```python
from build123d import *

# Parameters (mm, degrees)
SKETCH1_W           = 60
SKETCH1_H           = 30
BOSS_EXTRUDE1_DEPTH = 20
SKETCH2_W           = 37.506064646
SKETCH2_H           = 6.251724505
BOSS_EXTRUDE2_DEPTH = 5
BOSS_EXTRUDE3_DEPTH = 1


with BuildPart() as part:
    # Sketch1 → Boss-Extrude1 (new body)
    with BuildSketch(Plane(origin=(0, 0, 0), x_dir=(1, 0, 0), z_dir=(0, 1, 0))):
        Rectangle(SKETCH1_W, SKETCH1_H)
    extrude(amount=BOSS_EXTRUDE1_DEPTH)

    # Sketch2 → Boss-Extrude2 (add)
    with BuildSketch(Plane(origin=(0, 0, -15), x_dir=(-1, 0, 0), z_dir=(0, 0, -1))):
        with Locations((0, 9.939278845)):
            Rectangle(SKETCH2_W, SKETCH2_H)
    extrude(amount=BOSS_EXTRUDE2_DEPTH)

    # Sketch3 → Boss-Extrude3 (add)
    with BuildSketch(Plane.XZ):
        with BuildLine():
            Line((-30, 7.472956379), (-30, -8.939791774))
            ThreePointArc((-30, -8.939791774), (-38.206374076, -0.733417697), (-30, 7.472956379))
        make_face()
        with BuildLine():
            Line((30, 7.472956379), (30, -8.939791774))
            ThreePointArc((30, -8.939791774), (38.206374076, -0.733417697), (30, 7.472956379))
        make_face()
        with BuildLine():
            Line((-19.626363832, 15), (21.109917151, 15))
            Line((21.109917151, 15), (21.109917151, 16.556070662))
            ThreePointArc((21.109917151, 16.556070662), (19.645451057, 20.091604568), (16.109917151, 21.556070662))
            Line((16.109917151, 21.556070662), (-14.626363832, 21.556070662))
            ThreePointArc((-14.626363832, 21.556070662), (-18.161897738, 20.091604568), (-19.626363832, 16.556070662))
            Line((-19.626363832, 16.556070662), (-19.626363832, 15))
        make_face()
    extrude(amount=-BOSS_EXTRUDE3_DEPTH)


solid = part.part
```
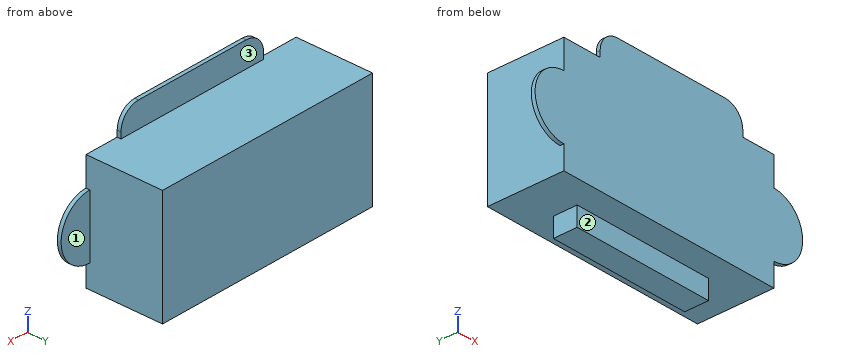
Design review of the part built by this model. Coordinates are the model's own, in mm. Face numbers are marked on the shaded views. A direction names the side the tool comes from. Give positions to 0.01 mm unless a question says otherwise; leave off trailing zeros. Write each loop counter-clockwise with the first axis right and the second up, starting at its lowest first coordinate (ties: lowest second). Pieces come first, ordered by that corner, then holes. Notation, with made-up numbers: (-6, 79) - (24, 79) arc R36 cw to (24, 114) - close; hole circle Ø2 at (-12.5, 75). An arc over 180 degrees is marked (long way). Return JSON: item names as keys, results as strings. Group by question number.
(1) Insertion check: pin 1 (2.5 mm diameter, centred on x = -3.5, z = -17.5, fed in from +Y); pin 2 (6 mm diameter, centred on y = 12.5, z = -4.5, fed in from +X); pin 3 (10 mm diameter, centred on y = 8.5, z = -4.5, fed in from -X). Each pin has a flat end and moves straight along its axis. Give the tip position at first contact, or say it passes through.
(2) We need section A-A, the plane y = 11. Give the boundary of the cut face in (x, z), then the cut area to 3 significant figures.
(3) Machinability: for the marked faces 1, 2 and 3, which of the approach directions +Z, -Z, +X, -X, +Y, -Y give a long, thin tool a straight path to every point of the face, cutting with its end or side? Answer none if there is none.
(4) We need section C-C, the plane z = 2.5. Give the boundary of the cut face in (x, y), then the cut area to 3 significant figures.
(5) We need section B-B, the plane x = 18. Give the boundary of the cut face in (y, z), then the cut area to 3 significant figures.
(6) We need section D-D, the plane y = 2.75. Give the boundary of the cut face in (x, z).
(7) To check wall thickness, follow probe 1 along Z at (x, y) = (-20, 3); probe 2 along X at (y, z) = (1.75, 6); probe 3 along Y at (x, z) = (19, 20.5). State the ranges of each line that lie inside material, in increasing order.
Reported:
{
 "1": {"pin 1": "stops at y = 13.07", "pin 2": "stops at x = 30", "pin 3": "stops at x = -30"},
 "2": {"outline": "(-30, -15) - (-18.75, -15) - (-18.75, -20) - (18.75, -20) - (18.75, -15) - (30, -15) - (30, 15) - (-30, 15) - close", "area": "1,990 mm2"},
 "3": {"face 1": "+Z, -Z, +X, +Y", "face 2": "-Z, +X, -X, -Y", "face 3": "+Z, +X, -X, +Y"},
 "4": {"outline": "(-37.54, 0) - (37.54, 0) - (37.54, 1) - (30, 1) - (30, 20) - (-30, 20) - (-30, 1) - (-37.54, 1) - close", "area": "1,220 mm2"},
 "5": {"outline": "(0, -15) - (6.81, -15) - (6.81, -20) - (13.07, -20) - (13.07, -15) - (20, -15) - (20, 15) - (1, 15) - (1, 21.19) - (0, 21.19) - close", "area": "637 mm2"},
 "6": {"outline": "(-30, -15) - (30, -15) - (30, 15) - (-30, 15) - close"},
 "7": {"probe 1": "z = -15 to 15", "probe 2": "x = -30 to 30", "probe 3": "y = 0 to 1"}
}
